Here's the drawing with two shaded views (mm, measured from the low corner). I have some questions. Round coordinates to 2 decimals unless told otherwise and drop trailing zeros. Loops run counter-clockwise (first coordinate to the right, second up) from the corner with the lowest first, then second, coordinate; pieces in that order, holes last. Notation, with made-up numbers: M -20,-8.75 L 12,-8.75 A30 cw 12,18.25 Z; hole C 10,-21 d6. An arc over 180 degrees is marked long. Answer as a JSON object with one key per item and string values.
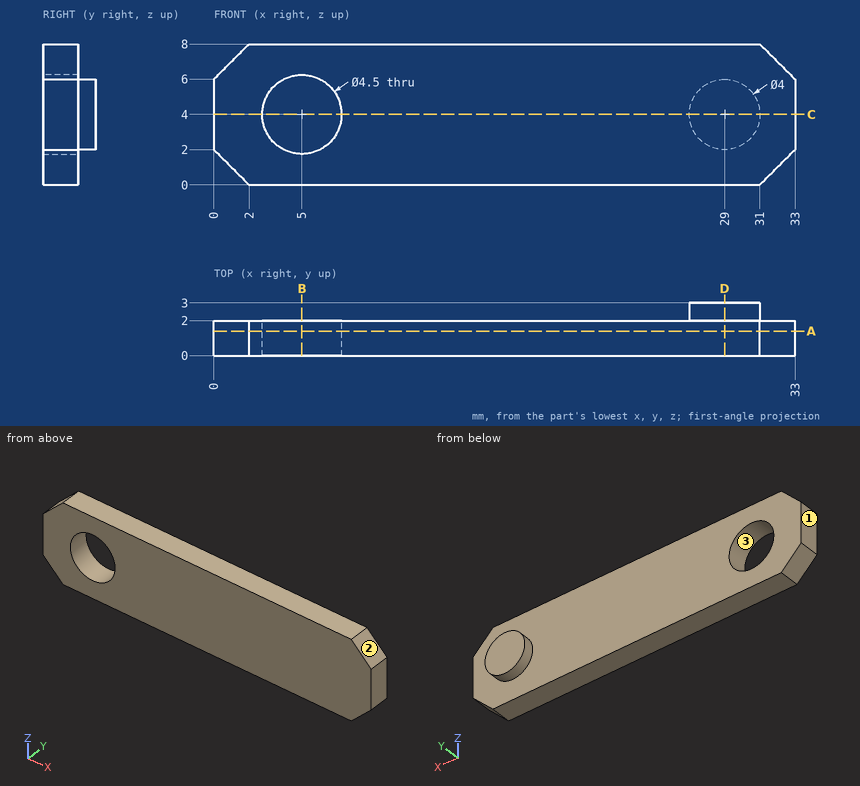
Item 1: We'd pull the mould along X, two halves only. Please class the marked faces 1, 2 and 3: +X half, -X half, draft (parallel to the pull), parting line (faces both ways), or undercut.
Solution:
{"face 1": "-X half", "face 2": "+X half", "face 3": "undercut"}
Item 2: I want a section at A-A on y = 1.4. List the corners of the cut face in (x, z) for me, plus the area to 3 significant figures.
Solution:
{"outline": "M 0,2 L 2,0 L 31,0 L 33,2 L 33,6 L 31,8 L 2,8 L 0,6 Z; hole C 5,4 d4.5", "area": "240 mm2"}
Item 3: I want a section at C-C on z = 4. List the corners of the cut face in (x, y) for me.
Solution:
{"outline": "M 0,0 L 2.75,0 L 2.75,2 L 0,2 Z; M 7.25,0 L 33,0 L 33,2 L 31,2 L 31,3 L 27,3 L 27,2 L 7.25,2 Z"}
Item 4: For P1, Ø2.5, axis at x = 5, z = 4, coming from the +Y side; P2, Ø2.5, axis at x = 19, z = 4, coming from the +Y side, each with a flat end and sliding along its axis, tell me the tip position at first contact or that it passes through.
Solution:
{"P1": "passes through", "P2": "stops at y = 2"}
Item 5: If I drill on L1, parallel to X at y = 0.6, z = 4; L2, parallel to Y at x = 3, z = 6.25; L3, parallel to Z at x = 4.5, y = 1.6, over which ranges is the centre line in solid material (lowest first)? Write a range as from..to.
Solution:
{"L1": "x = 0..2.75, 7.25..33", "L2": "y = 0..2", "L3": "z = 0..1.81, 6.19..8"}
Item 6: I want a section at B-B on x = 5. List the corners of the cut face in (y, z) for me.
Solution:
{"outline": "M 0,0 L 2,0 L 2,1.75 L 0,1.75 Z; M 0,6.25 L 2,6.25 L 2,8 L 0,8 Z"}
Item 7: I want a section at D-D on x = 29. List the corners of the cut face in (y, z) for me.
Solution:
{"outline": "M 0,0 L 2,0 L 2,2 L 3,2 L 3,6 L 2,6 L 2,8 L 0,8 Z"}
